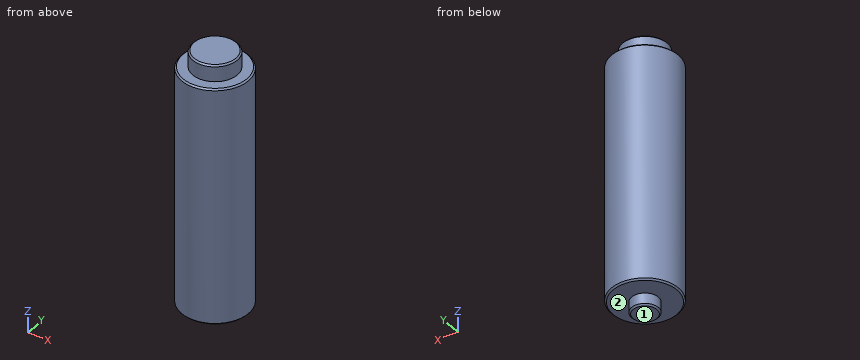
```python
from build123d import *

# Parameters (mm, degrees)
CHAMFER1_SIZE = 1


with BuildPart() as part:
    # Sketch1 → Revolve1 (revolve)
    with BuildSketch(Plane(origin=(0, 0, 0), x_dir=(0, 0, -1), z_dir=(1, 0, 0)), mode=Mode.PRIVATE) as revolve1_sk:
        Polygon((178, 0), (178, 9), (170, 9), (170, 22.5), (11, 22.5), (11, 15), (0, 15), (0, 0), align=None)
    revolve(revolve1_sk.sketch.rotate(Axis((0, 0, 0), (0, 0, -1)), 90), axis=Axis((0, 0, 0), (0, 0, -1)))

    # Chamfer1
    chamfer1_edges = [part.edges().sort_by_distance(p)[0] for p in [
        (-15, 0, 0),
        (-22.5, 0, -11),
        (-22.5, 0, -170),
        (-9, 0, -178),
    ]]
    chamfer(chamfer1_edges, length=CHAMFER1_SIZE)


solid = part.part
```
Geometry: final body of the model. Coordinates: model frame, mm. Face numbers are marked on the shaded views. A direction names the side the tool comes from. Round coordinates to 2 decimals unless told otherwise and drop trailing zeros. Order: outer loops, then holes, each group sorted by start corner. A loop starts at its lowest first (then second) coordinate and runs counter-clockwise, first axis right, second up. Notation, with made-up numbers: (63.25, 82) -> (67.25, 82) arc R22 cw to (67.25, 92) -> close; hole circle Ø3 at (-6, -7.75). An arc over 180 degrees is marked (long way). Use CSV: the item, a comma, the result in double quotes. Start each with the question number.
1) Section C-C (z = -78). Return the cut outline in (x, y), and give its area (3 significant figures).
2) Section A-A (x = 0). Return the cut outline in (y, z).
3) First-contact query: pin 1 Ø6 at (y, z) = (-15.5, -60.5) entering from -X; pin 2 Ø2 at (x, y) = (-14.5, 15.5) entering from -Z; pin 3 Ø4 at (x, z) = (0, -153.5) entering from +Y. Flat tips, straight axial feed; report the tip coordinate or a pass-through.
4) Material intervals for line 1 along Z through (x, y) = (-11, -8.5); line 2 along Z through (x, y) = (14.5, -13.5); line 3 along X through (y, z) = (-0.5, -25.5), sorted ascending. Write a range as from..to.
5) Set-up query: the marked faces 1 and 2. Return all of +Z, -Z, +X, -X, +Y, -Y with unobstructed straight access to the full face (end or side cutting, diameter ignored); none if empty.
Returned:
1,outline,"circle Ø45 at (0, 0)"
1,area,"1,590 mm²"
2,outline,"(-22.5, -169) -> (-21.5, -170) -> (-9, -170) -> (-9, -177) -> (-8, -178) -> (8, -178) -> (9, -177) -> (9, -170) -> (21.5, -170) -> (22.5, -169) -> (22.5, -12) -> (21.5, -11) -> (15, -11) -> (15, -1) -> (14, 0) -> (-14, 0) -> (-15, -1) -> (-15, -11) -> (-21.5, -11) -> (-22.5, -12) -> close"
3,pin 1,"stops at x = -18.71"
3,pin 2,"stops at z = -170"
3,pin 3,"stops at y = 22.5"
4,line 1,"z = -170..0"
4,line 2,"z = -170..-11"
4,line 3,"x = -22.49..22.49"
5,face 1,"-Z, +X, -X, +Y, -Y"
5,face 2,"-Z"
